from build123d import *

# Parameters (mm, degrees)
SKETCH1_W           = 20
SKETCH1_H           = 15
SKETCH1_R           = 1
BOSS_EXTRUDE1_DEPTH = 1
SKETCH2_W           = 6.421944946
SKETCH2_H           = 3.747416962
BOSS_EXTRUDE2_DEPTH = 5


with BuildPart() as part:
    # Sketch1 → Boss-Extrude1 (new body)
    with BuildSketch(Plane.XY):
        Rectangle(SKETCH1_W, SKETCH1_H)
        with Locations((-7, 4.5)):
            Circle(SKETCH1_R, mode=Mode.SUBTRACT)
        with Locations((-7, -2.5)):
            Circle(SKETCH1_R, mode=Mode.SUBTRACT)
        with Locations((7, 4.5)):
            Circle(SKETCH1_R, mode=Mode.SUBTRACT)
        with Locations((7, -2.5)):
            Circle(SKETCH1_R, mode=Mode.SUBTRACT)
    extrude(amount=BOSS_EXTRUDE1_DEPTH)

    # Sketch2 → Boss-Extrude2 (add)
    with BuildSketch(Plane.XY.offset(1)):
        with Locations((0, 5.626291519)):
            Rectangle(SKETCH2_W, SKETCH2_H)
    extrude(amount=BOSS_EXTRUDE2_DEPTH)


solid = part.part
Design review of the part built by this model. Coordinates are the model's own, in mm. A direction names the side the tool comes from. Round coordinates to 2 decimals unless told otherwise and drop trailing zeros. Loops run counter-clockwise (first coordinate to the right, second up) from the corner with the lowest first, then second, coordinate; pieces in that order, holes last. Notation, with made-up numbers: (-6.75, 67) - (49.25, 67) arc R18 ccw to (49.25, 88) - close; hole circle Ø6 at (0, 0.25). An arc over 180 degrees is marked (long way). One line per item, written item: value. Start each with the question number.
1) Consider section C-C on x = 7. Give the boundary of the cut face in (y, z).
2) Draft analysis for pull direction Y (two halves, no side actions). For faces 1 (the flat face through (0, 3.753, 3)), 2 (the flat face through (3.211, 6, 3)), 3 (the cylindrical face through (-7.13, 5.49, 0.49)), state which applies: +Y half, -Y half, draft (parallel to the pull), parting line (faces both ways), or undercut.
3) Consider section D-D on y = 4.5. Give the boundary of the cut face in (x, z).
4) Insertion check: pin 1 Ø1 at (x, z) = (0, 2.5) entering from -Y; pin 2 Ø3 at (y, z) = (4, 4) entering from +X; pin 3 Ø5 at (x, y) = (-6, 3) entering from +Z. Each pin has a flat end and moves straight along its axis. Give the tip position at first contact, or say it passes through.
5) Consider section B-B on z = 0.5. Give the boundary of the cut face in (x, y), then the cut area to 3 significant figures.
6) Consider section A-A on y = -2.5. Give the boundary of the cut face in (x, z).
7) To check wall thickness, follow L1, parallel to Y at x = -7, z = 0.55; L2, parallel to Y at x = -6.25, z = 0.5; L3, parallel to Y at x = 2.75, z = 1.3. State the ranges of each line that lie inside material, in increasing order. Write a range as from..to.
8) For faces 4 (the flat face through (-10, -0.1, 0.5)), 5 (the flat face through (-3.211, 6, 3)), list the 3-axis set-ups (+Z, -Z, +X, -X, +Y, -Y) from which the entire face can be reached by the end or side of a thin tool; tool diameter is ignored.
Reported:
1. outline: (-7.5, 0) - (-3.5, 0) - (-3.5, 1) - (-7.5, 1) - close; (-1.5, 0) - (3.5, 0) - (3.5, 1) - (-1.5, 1) - close; (5.5, 0) - (7.5, 0) - (7.5, 1) - (5.5, 1) - close
2. face 1: -Y half
2. face 2: draft
2. face 3: undercut
3. outline: (-10, 0) - (-8, 0) - (-8, 1) - (-10, 1) - close; (-6, 0) - (6, 0) - (6, 1) - (3.21, 1) - (3.21, 6) - (-3.21, 6) - (-3.21, 1) - (-6, 1) - close; (8, 0) - (10, 0) - (10, 1) - (8, 1) - close
4. pin 1: stops at y = 3.75
4. pin 2: stops at x = 3.21
4. pin 3: stops at z = 1
5. outline: (-10, -7.5) - (10, -7.5) - (10, 7.5) - (-10, 7.5) - close; hole circle Ø2 at (-7, -2.5); hole circle Ø2 at (-7, 4.5); hole circle Ø2 at (7, -2.5); hole circle Ø2 at (7, 4.5)
5. area: 287 mm^2
6. outline: (-10, 0) - (-8, 0) - (-8, 1) - (-10, 1) - close; (-6, 0) - (6, 0) - (6, 1) - (-6, 1) - close; (8, 0) - (10, 0) - (10, 1) - (8, 1) - close
7. L1: y = -7.5..-3.5, -1.5..3.5, 5.5..7.5
7. L2: y = -7.5..-3.16, -1.84..3.84, 5.16..7.5
7. L3: y = 3.75..7.5
8. face 4: +Z, -Z, -X, +Y, -Y
8. face 5: +Z, -X, +Y, -Y
